Build history of the part. All positions in model axes, mm. A direction names the side the tool comes from. Give positions to 0.01 mm unless a question says otherwise; leave off trailing zeros. Write each loop counter-clockwise with the first axis right and the second up, starting at its lowest first coordinate (ties: lowest second). Pieces come first, ordered by that corner, then holes. Notation, with made-up numbers: (86, -2) -> (92, -2) arc R24 ccw to (92, 36) -> close; hole circle Ø10 at (70, 77). An arc over 180 degrees is marked (long way). Put each result on its own line as item: value. Start each with the question number.
Item 1: Drill centre lines: line 1 along Y through (x, z) = (0, -9.25); line 2 along Z through (x, y) = (-12, 7). Where is each one in solid material? Low to high.
Item 2: Flat gauge pins, fed straight in: pin 1 Ø8 at (x, z) = (-9.5, -17.5) entering from +Y; pin 2 Ø4 at (y, z) = (-3, -16) entering from -X; pin 3 Ø12 at (y, z) = (10.5, -2.5) entering from +X. Where does each tip first touch, or does it go through?
Item 3: Tool access for faces 1 (the flat face through (6.5, 6.5, -20)), 2 (the flat face through (3.4, -12.3, -4)): list every direction of +Z, -Z, +X, -X, +Y, -Y with a clear straight run to the whole face (end or side of a thin tool).
Item 4: Two-plate mould, pull along X, no slides. Class faces 3 (the cylindrical face through (11.923, -3.755, -2.028)), 4 (the cylindrical face through (7.62, -3.16, -9.49)), 5 (the flat face through (-3, 8, 0)): pulls with the +X half, pulls with the -X half, needs draft (parallel to the pull), parting line crosses it, or undercut.
Item 5: Slice it at C-C, the plane z = -3.25. List the corners of the cut face in (x, y).
Item 6: Slice it at A-A, the plane y = 0. List the corners of the cut face in (x, z).
Item 7: Slice it at D-D, the plane y = -10.75. List the corners of the cut face in (x, z), plus the area to 3 significant figures.
```python
from build123d import *

# Parameters (mm, degrees)
M18X1_5_TAPPED_HOLE1_D     = 16.5
M18X1_5_TAPPED_HOLE1_DEPTH = 43.5
M18X1_5_TAPPED_HOLE1_TIP   = 4.957100107
CHAMFER1_SIZE              = 0.75


with BuildPart() as part:
    # Sketch1 → Revolve1 (revolve)
    with BuildSketch(Plane(origin=(0, 0, 0), x_dir=(1, 0, 0), z_dir=(0, 1, 0))):
        Polygon((7.5, 0), (12.5, 0), (12.5, 4), (15, 4), (15, 20), (7.5, 20), align=None)
    revolve(axis=Axis((0, 0, 0), (0, 0, -1)))

    # M18x1.5 Tapped Hole1
    with Locations(Plane(origin=(0, 0, -20), x_dir=(-1, 0, 0), z_dir=(0, 0, -1))):
        with Locations((0, 0)):
            Hole(M18X1_5_TAPPED_HOLE1_D / 2, depth=M18X1_5_TAPPED_HOLE1_DEPTH)
            with Locations((0, 0, -(M18X1_5_TAPPED_HOLE1_DEPTH + M18X1_5_TAPPED_HOLE1_TIP / 2))):  # 118° drill point
                Cone(0, M18X1_5_TAPPED_HOLE1_D / 2, M18X1_5_TAPPED_HOLE1_TIP, mode=Mode.SUBTRACT)

    # Chamfer1
    chamfer1_edges = [part.edges().sort_by_distance(p)[0] for p in [
        (-8.25, 0, -20),
    ]]
    chamfer(chamfer1_edges, length=CHAMFER1_SIZE)


solid = part.part
```
Values follow:
1. line 1: -15 to -8.25, 8.25 to 15
1. line 2: -20 to -4
2. pin 1: y = 13.96
2. pin 2: x = -14.97
2. pin 3: x = 14.25
3. face 1: -Z, +X, -X, +Y, -Y
3. face 2: +Z
4. face 3: parting line crosses it
4. face 4: undercut
4. face 5: needs draft
5. outline: circle Ø25 at (0, 0); hole circle Ø16.5 at (0, 0)
6. outline: (-15, -20) -> (-9, -20) -> (-8.25, -19.25) -> (-8.25, 0) -> (-12.5, 0) -> (-12.5, -4) -> (-15, -4) -> close; (8.25, -19.25) -> (9, -20) -> (15, -20) -> (15, -4) -> (12.5, -4) -> (12.5, 0) -> (8.25, 0) -> close
7. outline: (-10.46, -20) -> (10.46, -20) -> (10.46, -4) -> (6.38, -4) -> (6.38, 0) -> (-6.38, 0) -> (-6.38, -4) -> (-10.46, -4) -> close
7. area: 386 mm2
